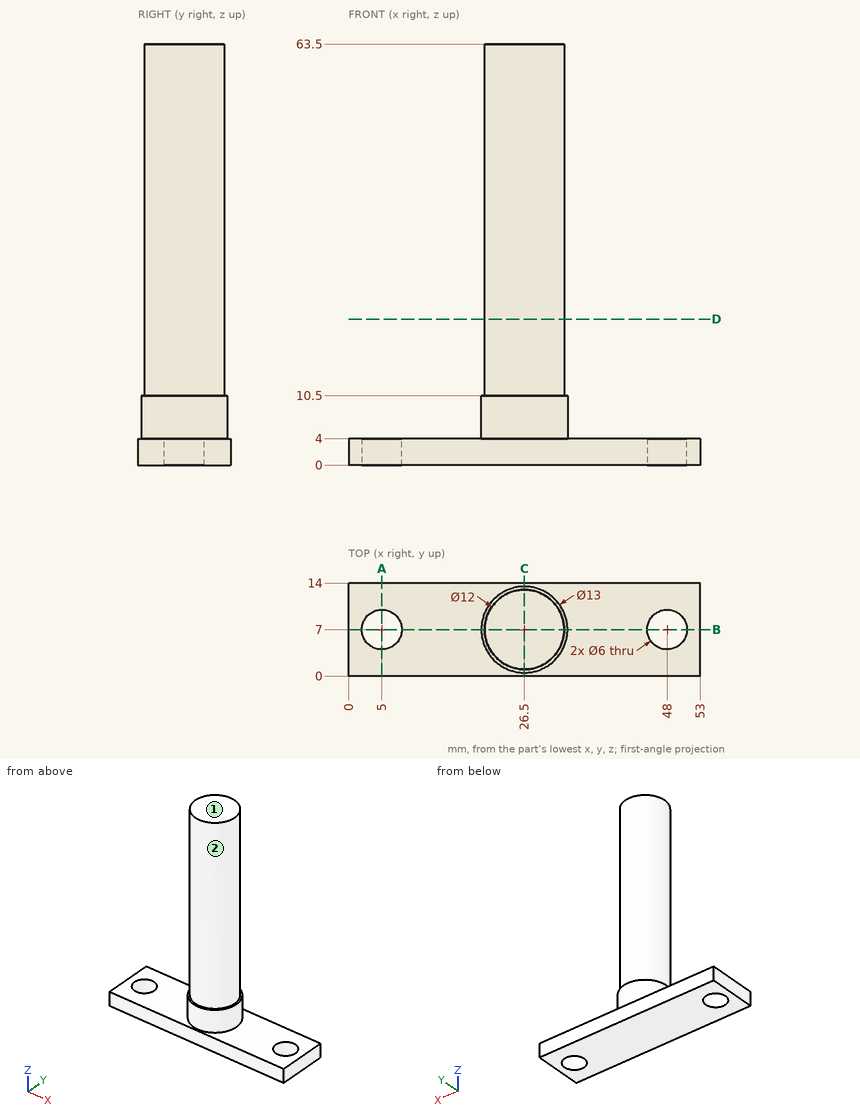
Study the drawing (mm; zero at the part's minimum x, y, z) and answer. A direction names the side the tool comes from. Give positions to 0.01 mm unless a question says otherwise; leave off trailing zeros. Loops run counter-clockwise (first coordinate to the right, second up) from the corner with the lowest first, then second, coordinate; pieces in that order, holes last. Notation, with made-up numbers: (-26, 23) -> (23, 23) arc R19 cw to (23, 45) -> close; hole circle Ø5 at (-13.5, 18). An arc over 180 degrees is marked (long way). Use a Markdown table: item, result. Add a question column.
1) Consider line 1 along Y through (x, z) = (5, 0.9); line 2 along Z through (x, y) = (8.5, 13); line 3 along X through (y, z) = (12, 17). Determine where each line is inside the solid, lowest interval first.
2) The part is cut by section B-B, the plane y = 7. Determine the outline of the cut face in (x, z).
3) The part is cut by section A-A, the plane x = 5. Determine the outline of the cut face in (y, z).
4) Each of these flat-tipped pins is pushed along its axis until it touches: P1, Ø1.5, axis at y = 9.5, z = 26.5, coming from the +X side; P2, Ø1.5, axis at x = 23, z = 39.5, coming from the +Y side; P3, Ø2, axis at x = 21, z = 8, coming from the +Y side. Where does it stop, or does it pass through?
5) The part is cut by section C-C, the plane x = 26.5. Determine the outline of the cut face in (y, z).
6) Which of the six approach directions +Z, -Z, +X, -X, +Y, -Y give full straight-line access (tool end or side, diameter ignored) to the marked faces 1 and 2?
7) The part is cut by section D-D, the plane z = 22. Determine the outline of the cut face in (x, y).
Reported:
| question | item | result |
|---|---|---|
| 1 | line 1 | y = 0 to 4, 10 to 14 |
| 1 | line 2 | z = 0 to 4 |
| 1 | line 3 | x = 23.18 to 29.82 |
| 2 | outline | (0, 0) -> (2, 0) -> (2, 4) -> (0, 4) -> close; (8, 0) -> (45, 0) -> (45, 4) -> (33, 4) -> (33, 10.5) -> (32.5, 10.5) -> (32.5, 63.5) -> (20.5, 63.5) -> (20.5, 10.5) -> (20, 10.5) -> (20, 4) -> (8, 4) -> close; (51, 0) -> (53, 0) -> (53, 4) -> (51, 4) -> close |
| 3 | outline | (0, 0) -> (4, 0) -> (4, 4) -> (0, 4) -> close; (10, 0) -> (14, 0) -> (14, 4) -> (10, 4) -> close |
| 4 | P1 | stops at x = 32.24 |
| 4 | P2 | stops at y = 12.33 |
| 4 | P3 | stops at y = 11.69 |
| 5 | outline | (0, 0) -> (14, 0) -> (14, 4) -> (13.5, 4) -> (13.5, 10.5) -> (13, 10.5) -> (13, 63.5) -> (1, 63.5) -> (1, 10.5) -> (0.5, 10.5) -> (0.5, 4) -> (0, 4) -> close |
| 6 | face 1 | +Z, +X, -X, +Y, -Y |
| 6 | face 2 | +Z |
| 7 | outline | circle Ø12 at (26.5, 7) |
